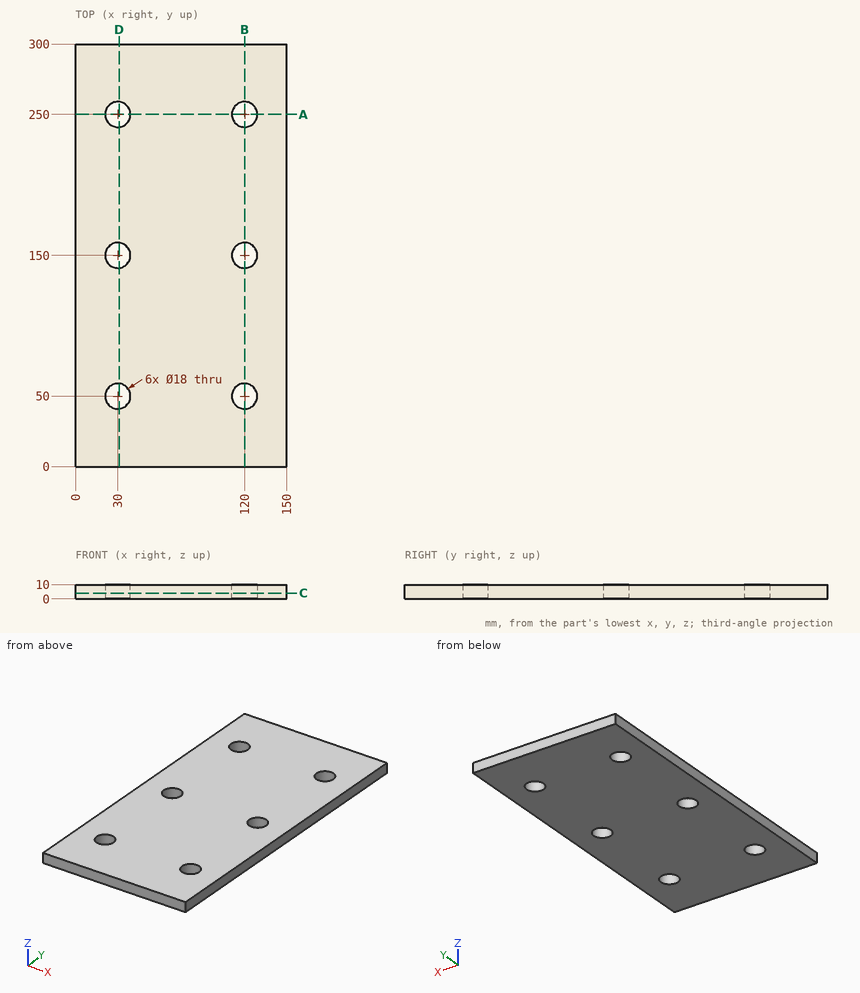
For this review, use the dimensioned drawing (mm, ordinates from the lowest corner) and the shaded views. Coordinates: 2 decimals unless noted, no trailing zeros. Write each loop counter-clockwise with the first axis right and the second up, starting at its lowest first coordinate (ties: lowest second). Pieces come first, ordered by that corner, then holes. Notation, with made-up numbers: (-32, 46.25) - (-24, 46.25) arc R17 cw to (-24, 63.25) - close; hole circle Ø10 at (66.25, 70.5). An arc over 180 degrees is marked (long way). Answer in a Markdown table with one row per item. Add a question column.
Q1. Consider section A-A on y = 250. Give the boundary of the cut face in (x, z).
Q2. Consider section C-C on z = 4. Give the boundary of the cut face in (x, y), then the cut area to 3 significant figures.
Q3. To check wall thickness, follow line 1 along Y through (x, z) = (120, 3.5); line 2 along X through (y, z) = (150.5, 6); line 3 along X through (y, z) = (253.5, 1.25). State the ranges of each line that lie inside material, in increasing order. Write a range as from..to.
Q4. Clearance check with flat-ended pins moving along their axes: pin 1 (5 mm diameter, centred on x = 47, z = 5.5, fed in from -Y); pin 2 (16 mm diameter, centred on x = 30, y = 250, fed in from -Z). State where each tip first meets the part, or that it passes through.
Q5. Consider section B-B on x = 120. Give the boundary of the cut face in (y, z).
Q6. Consider section D-D on x = 31. Give the boundary of the cut face in (y, z).
Answers below:
| question | item | result |
|---|---|---|
| 1 | outline | (0, 0) - (21, 0) - (21, 10) - (0, 10) - close; (39, 0) - (111, 0) - (111, 10) - (39, 10) - close; (129, 0) - (150, 0) - (150, 10) - (129, 10) - close |
| 2 | outline | (0, 0) - (150, 0) - (150, 300) - (0, 300) - close; hole circle Ø18 at (30, 50); hole circle Ø18 at (30, 150); hole circle Ø18 at (30, 250); hole circle Ø18 at (120, 50); hole circle Ø18 at (120, 150); hole circle Ø18 at (120, 250) |
| 2 | area | 43,500 mm² |
| 3 | line 1 | 0..41, 59..141, 159..241, 259..300 |
| 3 | line 2 | 0..21.01, 38.99..111.01, 128.99..150 |
| 3 | line 3 | 0..21.71, 38.29..111.71, 128.29..150 |
| 4 | pin 1 | y = 0 |
| 4 | pin 2 | through |
| 5 | outline | (0, 0) - (41, 0) - (41, 10) - (0, 10) - close; (59, 0) - (141, 0) - (141, 10) - (59, 10) - close; (159, 0) - (241, 0) - (241, 10) - (159, 10) - close; (259, 0) - (300, 0) - (300, 10) - (259, 10) - close |
| 6 | outline | (0, 0) - (41.06, 0) - (41.06, 10) - (0, 10) - close; (58.94, 0) - (141.06, 0) - (141.06, 10) - (58.94, 10) - close; (158.94, 0) - (241.06, 0) - (241.06, 10) - (158.94, 10) - close; (258.94, 0) - (300, 0) - (300, 10) - (258.94, 10) - close |
